Read the model definition and answer for the solid it produces. Units are mm, in the model's axes. Face numbers are marked on the shaded views. A direction names the side the tool comes from. Give positions to 0.01 mm unless a question says otherwise; leave off trailing zeros. Loops run counter-clockwise (first coordinate to the right, second up) from the corner with the lowest first, then second, coordinate; pieces in that order, holes last. Notation, with made-up numbers: (84, 12) - (102, 12) arc R15 ccw to (102, 24) - close; hole circle Ø3 at (-13, -17.75). An arc over 180 degrees is marked (long way). Write item = value, one per line. Start each with the question number.
from build123d import *

# Parameters (mm, degrees)
BASE_BLOCK_DEPTH          = 50
BODY_RECESS_CUT_DEPTH     = 50
BEARING_HUB_PROFILE_R     = 40
BEARING_HUB_BOSS_DEPTH    = 50
HUB_START                 = 5
HUB_FLANGE_PROFILE_R      = 40
HUB_FLANGE_BOSS_DEPTH     = 5
MAIN_BORE_PROFILE_R       = 28
MAIN_BORE_CUT_DEPTH       = 113
TOP_SLOT_PROFILE_W        = 30
TOP_SLOT_PROFILE_H        = 100
TOP_SLOT_CUT_DEPTH        = 10
SIDE_ARM_BOSS_DEPTH       = 40
ARM_HOLE_PROFILE_R        = 28
ARM_HOLE_CUT_DEPTH        = 15
SHAFT_HUB_BOSS_DEPTH      = 5
SHAFT_HUB_BOSS_DEPTH_BACK = 15
SHAFT_HUB_PROFILE_R       = 28
KEYED_BORE_CUT_DEPTH      = 30
REAR_RING_PROFILE_R       = 40
REAR_RING_BOSS_DEPTH      = 5
THROUGH_BORE_PROFILE_R    = 28
THROUGH_BORE_CUT_DEPTH    = 194
SECOND_SLOT_PROFILE_W     = 30
SECOND_SLOT_PROFILE_H     = 100
SECOND_SLOT_CUT_DEPTH     = 10


with BuildPart() as part:
    # Base Block Profile → Base Block (new body)
    with BuildSketch(Plane(origin=(0, 0, 0), x_dir=(0, 0, -1), z_dir=(1, 0, 0))):
        Polygon((50, 0), (50, 53), (-50, 53), (-50, -53), (50, -53), align=None)
    extrude(amount=-BASE_BLOCK_DEPTH)

    # Body Recess Profile → Body Recess Cut (cut)
    with BuildSketch(Plane(origin=(0, 0, 0), x_dir=(0, 0, -1), z_dir=(1, 0, 0))):
        with BuildLine():
            Line((-50, 0), (-50, 22.5))
            Line((-50, 22.5), (-33.071891388, 22.5))
            ThreePointArc((-33.071891388, 22.5), (40, 0), (-33.071891388, -22.5))
            Line((-33.071891388, -22.5), (-50, -22.5))
            Line((-50, -22.5), (-50, 0))
        make_face()
    extrude(amount=-BODY_RECESS_CUT_DEPTH, mode=Mode.SUBTRACT)

    # Bearing Hub Profile → Bearing Hub Boss (add)
    with BuildSketch(Plane(origin=(0, 0, 0), x_dir=(0, 0, -1), z_dir=(1, 0, 0))):
        Circle(BEARING_HUB_PROFILE_R)
    extrude(amount=-BEARING_HUB_BOSS_DEPTH)

    # Hub Flange Profile → Hub Flange Boss (add)
    with BuildSketch(Plane(origin=(0, 0, 0), x_dir=(0, 0, -1), z_dir=(1, 0, 0)).offset(HUB_START)):
        Circle(HUB_FLANGE_PROFILE_R)
    extrude(amount=-HUB_FLANGE_BOSS_DEPTH)

    # Main Bore Profile → Main Bore Cut (cut)
    with BuildSketch(Plane(origin=(5, 0, 0), x_dir=(0, 0, -1), z_dir=(1, 0, 0))):
        Circle(MAIN_BORE_PROFILE_R)
    extrude(amount=-MAIN_BORE_CUT_DEPTH, mode=Mode.SUBTRACT)

    # Top Slot Profile → Top Slot Cut (cut)
    with BuildSketch(Plane(origin=(0, 53, 0), x_dir=(1, 0, 0), z_dir=(0, 1, 0))):
        with Locations((-25, 0)):
            Rectangle(TOP_SLOT_PROFILE_W, TOP_SLOT_PROFILE_H)
    extrude(amount=-TOP_SLOT_CUT_DEPTH, mode=Mode.SUBTRACT)

    # Side Arm Profile → Side Arm Boss (add)
    with BuildSketch(Plane(origin=(-5, 0, 0), x_dir=(0, 0, -1), z_dir=(1, 0, 0))):
        Polygon((-90, 0), (-90, 35), (-50, 35), (-50, 22.5), (-75, 22.5), (-75, -22.5), (-50, -22.5), (-50, -35), (-90, -35), align=None)
    extrude(amount=-SIDE_ARM_BOSS_DEPTH)

    # Arm Hole Profile → Arm Hole Cut (cut)
    with BuildSketch(Plane.XY.offset(90)):
        with Locations((-25, 0)):
            Circle(ARM_HOLE_PROFILE_R)
    extrude(amount=-ARM_HOLE_CUT_DEPTH, mode=Mode.SUBTRACT)

    # Shaft Hub Profile → Shaft Hub Boss (add, two sides: drawn at the far end of the back side and taken through both)
    with BuildSketch(Plane.XY.offset(90).offset(-SHAFT_HUB_BOSS_DEPTH_BACK)):
        with Locations((-25, 0)):
            Circle(SHAFT_HUB_PROFILE_R)
    extrude(amount=SHAFT_HUB_BOSS_DEPTH + SHAFT_HUB_BOSS_DEPTH_BACK)

    # Keyed Bore Profile → Keyed Bore Cut (cut)
    with BuildSketch(Plane.XY.offset(95)):
        with BuildLine():
            Line((-21, 13.416407865), (-21, 17))
            Line((-21, 17), (-29, 17))
            Line((-29, 17), (-29, 13.416407865))
            ThreePointArc((-29, 13.416407865), (-25, -14), (-21, 13.416407865))
        make_face()
    extrude(amount=-KEYED_BORE_CUT_DEPTH, mode=Mode.SUBTRACT)

    # Rear Ring Profile → Rear Ring Boss (add)
    with BuildSketch(Plane.ZY.offset(50)):
        with Locations(Location((0, 0, 0), (0, 0, 180))):
            Circle(REAR_RING_PROFILE_R)
    extrude(amount=REAR_RING_BOSS_DEPTH)

    # Through Bore Profile → Through Bore Cut (cut)
    with BuildSketch(Plane(origin=(5, 0, 0), x_dir=(0, 0, -1), z_dir=(1, 0, 0))):
        Circle(THROUGH_BORE_PROFILE_R)
    extrude(amount=-THROUGH_BORE_CUT_DEPTH, mode=Mode.SUBTRACT)

    # Second Slot Profile → Second Slot Cut (cut)
    with BuildSketch(Plane.XZ.offset(53)):
        with Locations((-25, 0)):
            Rectangle(SECOND_SLOT_PROFILE_W, SECOND_SLOT_PROFILE_H)
    extrude(amount=-SECOND_SLOT_CUT_DEPTH, mode=Mode.SUBTRACT)


solid = part.part
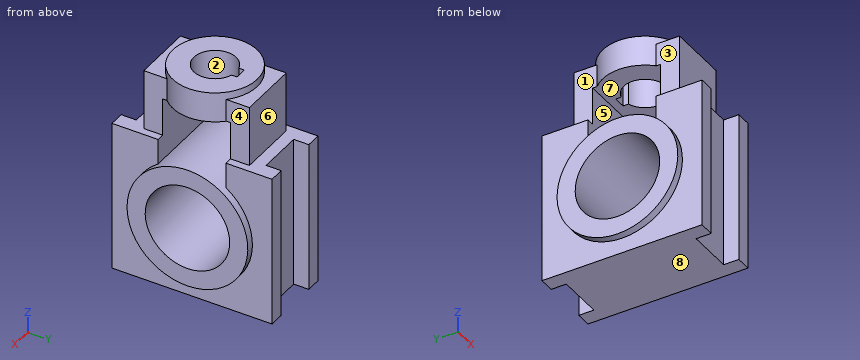
1. Given P1, Ø6, axis at x = -18, z = 39, coming from the -Y side; P2, Ø25, axis at x = -25, y = 0, coming from the +Z side; P3, Ø3, axis at y = -50.5, z = 22.5, coming from the -X side, each flat-ended and moving along its own axis, determine where each tip first touches the part or whether it passes through.
2. For a pull along Y with two mould halves and no side action, classify the marked faces 6, 7 and 8 as released by +Y, released by -Y, zero draft, split by the parting line, or undercut.
3. A cutting plane is placed at A-A on y = 0. Give the vertices of the cut face in (x, z), and give its area (3 significant figures).
4. A cutting plane is placed at C-C on x = -25. Give the vertices of the cut face in (y, z).
5. A cutting plane is placed at B-B on z = 79.5. Give the vertices of the cut face in (x, y), and give its area (3 significant figures).
6. Consider line 1 along Y through (x, z) = (-19, 0); line 2 along Z through (x, y) = (-6, 4.5); line 3 along Y through (x, z) = (-26, 63.5). Determine where each line is inside the solid, lowest interval first. Write a range as [from, to].
7. A tool of negligible diameter and unlimited length cuts with its end or side. For the marked faces 1, 2, 3, 4 and 5, from which of +Z, -Z, +X, -X, +Y, -Y can it reach the whole face along a straight path? Write none if from no direction.
8. A cutting plane is placed at D-D on z = 54. Give the vertices of the cut face in (x, y).
Reply:
q1.P1 = -43
q1.P2 = 40
q1.P3 = -50
q2.face_6 = released by +Y
q2.face_7 = undercut
q2.face_8 = zero draft
q3.outline = (-55, -40) - (-50, -40) - (-50, -50) - (0, -50) - (0, -40) - (5, -40) - (5, -28) - (-55, -28) - close; (-55, 28) - (5, 28) - (5, 40) - (-55, 40) - close; (-53, 75) - (-39, 75) - (-39, 95) - (-53, 95) - close; (-11, 75) - (3, 75) - (3, 95) - (-11, 95) - close
q3.area = 2,500 mm^2
q4.outline = (-43, -50) - (43, -50) - (43, 50) - (35, 50) - (35, 90) - (28, 90) - (28, 95) - (17, 95) - (17, 75) - (22.5, 75) - (22.5, 33.07) arc R40 ccw to (-22.5, 33.07) - (-22.5, 75) - (-14, 75) - (-14, 95) - (-28, 95) - (-28, 90) - (-35, 90) - (-35, 50) - (-43, 50) - close; hole circle Ø56 at (0, 0)
q5.outline = (-45, -35) - (-5, -35) - (-5, -19.6) arc R28 ccw to (-5, 19.6) - (-5, 35) - (-45, 35) - (-45, 19.6) arc R28 ccw to (-45, -19.6) - close; hole (-29, 13.42) arc R14 ccw (long way) to (-21, 13.42) - (-21, 17) - (-29, 17) - close
q5.area = 2,590 mm^2
q6.line_1 = [-43, -28], [28, 43]
q6.line_2 = [-50, -27.64], [27.64, 39.75], [75, 95]
q6.line_3 = [-35, -22.5], [22.5, 35]
q7.face_1 = +Z, -X, +Y
q7.face_2 = +Z
q7.face_3 = +Z, -X, -Y
q7.face_4 = +Z, +X, +Y
q7.face_5 = +X, -X
q8.outline = (-45, -35) - (-5, -35) - (-5, -22.5) - (-45, -22.5) - close; (-45, 22.5) - (-5, 22.5) - (-5, 35) - (-45, 35) - close
